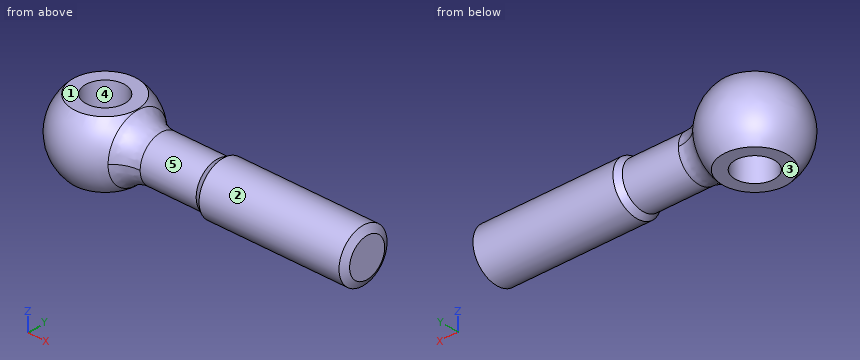
```python
from build123d import *
from build123d.topology import SkipClean

# Parameters (mm, degrees)
CUT_EXTRUDE1_DEPTH      = 13.124356
CUT_EXTRUDE1_DEPTH_BACK = 13.124356
SKETCH4_R               = 3
CUT_EXTRUDE2_DEPTH      = 16.556349
CHAMFER1_SIZE           = 0.4
FILLET1_R               = 5


with BuildPart() as part:
    # Sketch1 → Boss-Revolve (revolve)
    with BuildSketch(Plane.XY):
        with BuildLine():
            Line((-7, 0), (7, 0))
            ThreePointArc((7, 0), (0, 7), (-7, 0))
        make_face()
    revolve(axis=Axis((-13.286843, 0, 0), (1, 0, 0)))

    # Sketch2 → Cut-Extrude1 (cut, two sides: drawn at the far end of the back side and taken through both)
    with SkipClean():  # the faces are left unmerged after this step: merging them gives an invalid solid
        with BuildSketch(Plane(origin=(0, 0, 0), x_dir=(0, 0, -1), z_dir=(1, 0, 0)).offset(-CUT_EXTRUDE1_DEPTH_BACK)):
            with BuildLine():
                Line((-5, 4.898979), (-5, -4.898979))
                ThreePointArc((-5, -4.898979), (-7, 0), (-5, 4.898979))
            make_face()
            with BuildLine():
                Line((5, 4.898979), (5, -4.898979))
                ThreePointArc((5, -4.898979), (7, 0), (5, 4.898979))
            make_face()
        extrude(amount=CUT_EXTRUDE1_DEPTH + CUT_EXTRUDE1_DEPTH_BACK, mode=Mode.SUBTRACT)

    # Sketch4 → Cut-Extrude2 (cut, through all)
    with SkipClean():  # the faces are left unmerged after this step: merging them gives an invalid solid
        with BuildSketch(Plane.XY.offset(5)):
            Circle(SKETCH4_R)
        extrude(amount=-CUT_EXTRUDE2_DEPTH, mode=Mode.SUBTRACT)

    # Sketch5 → Boss-Revolve1 (revolve)
    with SkipClean():  # the faces are left unmerged after this step: merging them gives an invalid solid
        with BuildSketch(Plane.XY, mode=Mode.PRIVATE) as boss_revolve1_sk:
            Polygon((3.469445, 3.45875), (3.469445, 0), (40, 0), (40, 4), (18, 4), (17.062528, 3.45875), align=None)
        revolve(boss_revolve1_sk.sketch.rotate(Axis((0, 0, 0), (1, 0, 0)), 180), axis=Axis((0, 0, 0), (1, 0, 0)))

    # Chamfer1
    chamfer1_edges = [part.edges().sort_by_distance(p)[0] for p in [
        (40, 4, 0),
    ]]
    chamfer(chamfer1_edges, length=CHAMFER1_SIZE)

    # Sketch6 → Cut-Revolve1 (revolve, cut)
    with SkipClean():  # the faces are left unmerged after this step: merging them gives an invalid solid
        with BuildSketch(Plane.XY, mode=Mode.PRIVATE) as cut_revolve1_sk:
            Polygon((39.375018, 4), (40.624982, 4), (40, 2.9175), align=None)
        revolve(cut_revolve1_sk.sketch.rotate(Axis((0, 0, 0), (1, 0, 0)), 180), axis=Axis((0, 0, 0), (1, 0, 0)), mode=Mode.SUBTRACT)

    # Fillet1
    fillet1_edges = [part.edges().sort_by_distance(p)[0] for p in [
        (6.085807, 0, -3.45875),
    ]]
    fillet(fillet1_edges, radius=FILLET1_R)


solid = part.part
```
For this review, take the finished solid that the model builds, in its own axes (mm). Face numbers are marked on the shaded views. A direction names the side the tool comes from. Round coordinates to 2 decimals unless told otherwise and drop trailing zeros. Order: outer loops, then holes, each group sorted by start corner. A loop starts at its lowest first (then second) coordinate and runs counter-clockwise, first axis right, second up.
Q1. We need section C-C, the plane y = -6. Give the boundary of the cut face in (x, z).
Findings below:
outline: circle Ø7.21 at (0, 0)
Q2. We need section A-A, the plane x = -2.5. Give the boundary of the cut face in (y, z).
Findings below:
outline: (-4.21, -5) - (-1.66, -5) - (-1.66, 5) - (-4.21, 5) arc R6.54 ccw to start; (1.66, -5) - (4.21, -5) arc R6.54 ccw to (4.21, 5) - (1.66, 5) - close
Q3. Machinability: for the marked faces 1 and 2, which of the approach directions +Z, -Z, +X, -X, +Y, -Y give a long, thin tool a straight path to every point of the face, cutting with its end or side? Answer none if there is none.
Findings below:
face 1: +Z, +X, -X, +Y, -Y
face 2: +X
Q4. Wall thickness on line 1 (Y direction, x = 0, z = 3.25); line 2 (Y direction, x = 0, z = -2.5); line 3 (X direction, y = 2.5, z = -4): over which ranges is each line inside the solid? List them lowest first.
Findings below:
line 1: y = -6.2 to -3, 3 to 6.2
line 2: y = -6.54 to -3, 3 to 6.54
line 3: x = -5.17 to -1.66, 1.66 to 5.2
Q5. Mouldability with a two-part tool opening along Y and no side actions: class the marked faces 3, 4 and 5 as pulls with the +Y half, pulls with the -Y half, needs draft (parallel to the pull), parting line crosses it, or undercut.
Findings below:
face 3: needs draft
face 4: undercut
face 5: parting line crosses it
Q6. We need section B-B, the plane x = 11.5. Give the boundary of the cut face in (y, z).
Findings below:
outline: circle Ø6.92 at (0, 0)
Q7. Insertion check: P1, Ø1, axis at x = 29.5, y = 1.5, coming from the -Z side; P2, Ø8, axis at x = 22, y = -2, coming from the +Z side; P3, Ø2, axis at x = 30, y = -4.5, coming from the +Z side. Each pin has a flat end and moves straight along its axis. Give the tip position at first contact, or say it passes through.
Findings below:
P1: stops at z = -3.87
P2: stops at z = 4
P3: stops at z = 1.94
